Read the model definition and answer for the solid it produces. Units are mm, in the model's axes. Give positions to 0.01 mm unless a question says otherwise; leave off trailing zeros. Order: outer loops, then holes, each group sorted by start corner. A loop starts at its lowest first (then second) coordinate and runs counter-clockwise, first axis right, second up. Notation, with made-up numbers: (-30.5, 50.25) - (6.5, 50.25) arc R20 ccw to (6.5, 70.25) - close; hole circle Ø9 at (6.5, 1.5). An arc over 180 degrees is marked (long way). Use a Markdown table: item, result. Add a question column.
1. A cutting plane is placed at C-C on y = -22.5. Determine the outline of the cut face in (x, z).
2. A cutting plane is placed at B-B on y = -14. Determine the outline of the cut face in (x, z).
3. A cutting plane is placed at D-D on x = 8.5. Determine the outline of the cut face in (y, z).
4. A flat-ended cylindrical pin translates along its axis: P1, Ø0.6, axis at y = -22.5, z = 1.5, coming from the +X side. Find the tip coordinate at first contact, or state that the pin passes through.
5. A cutting plane is placed at A-A on z = 1.65. Determine the outline of the cut face in (x, y), and give its area (3 significant figures).
6. Consider L1, parallel to Y at x = 8.5, z = 1.55; L2, parallel to X at y = -17, z = 1.85; L3, parallel to Y at x = 6, z = 1.95. Determine where each line is inside the solid, lowest interval first.
```python
from build123d import *

# Parameters (mm, degrees)
SKETCH_1_R      = 2
EXTRUDE_1_DEPTH = 2


with BuildPart() as part:
    # 草图1 → 凸台-拉伸1 (new body)
    with BuildSketch(Plane.XY):
        with BuildLine():
            Line((-14.576201266, -23.207463353), (-15.742490369, -16.580463555))
            ThreePointArc((-15.742490369, -16.580463555), (-15.927700406, -16.024070615), (-16.26632367, -15.545311649))
            ThreePointArc((-16.26632367, -15.545311649), (0, 22.5), (16.26632367, -15.545311649))
            ThreePointArc((16.26632367, -15.545311649), (15.927700406, -16.024070615), (15.742490369, -16.580463555))
            Line((15.742490369, -16.580463555), (14.576201266, -23.207463353))
            ThreePointArc((14.576201266, -23.207463353), (14.420792767, -23.592708818), (14.122248494, -23.881563776))
            ThreePointArc((14.122248494, -23.881563776), (8.541490175, -26.531326793), (2.5, -27.822258212))
            Line((2.5, -27.822258212), (2.5, -19.67030278))
            ThreePointArc((2.5, -19.67030278), (0, 17.16), (-2.5, -19.67030278))
            Line((-2.5, -19.67030278), (-2.5, -27.822258212))
            ThreePointArc((-2.5, -27.822258212), (-8.541490175, -26.531326793), (-14.122248494, -23.881563776))
            ThreePointArc((-14.122248494, -23.881563776), (-14.420792767, -23.592708818), (-14.576201266, -23.207463353))
        make_face()
        with Locations((-8.5, -22.5)):
            Circle(SKETCH_1_R, mode=Mode.SUBTRACT)
        with Locations((8.5, -22.5)):
            Circle(SKETCH_1_R, mode=Mode.SUBTRACT)
    extrude(amount=EXTRUDE_1_DEPTH)


solid = part.part
```
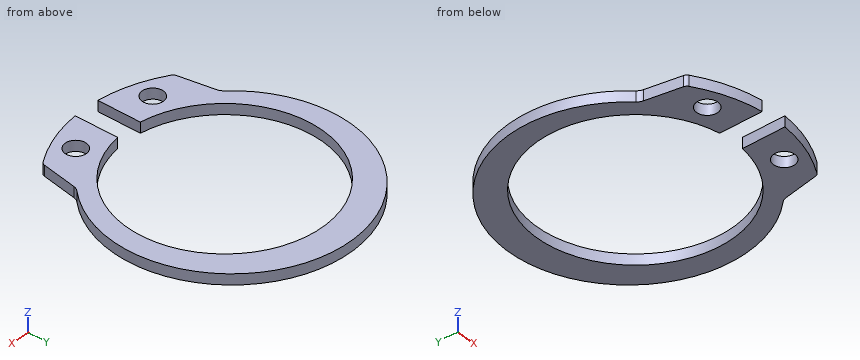
Output values:
| question | item | result |
|---|---|---|
| 1 | outline | (-14.7, 0) - (-10.5, 0) - (-10.5, 2) - (-14.7, 2) - close; (-6.5, 0) - (-2.5, 0) - (-2.5, 2) - (-6.5, 2) - close; (2.5, 0) - (6.5, 0) - (6.5, 2) - (2.5, 2) - close; (10.5, 0) - (14.7, 0) - (14.7, 2) - (10.5, 2) - close |
| 2 | outline | (-17.61, 0) - (-13.49, 0) - (-13.49, 2) - (-17.61, 2) - close; (13.49, 0) - (17.61, 0) - (17.61, 2) - (13.49, 2) - close |
| 3 | outline | (-26.55, 0) - (-24.5, 0) - (-24.5, 2) - (-26.55, 2) - close; (-20.5, 0) - (-17.77, 0) - (-17.77, 2) - (-20.5, 2) - close; (15.09, 0) - (20.83, 0) - (20.83, 2) - (15.09, 2) - close |
| 4 | P1 | x = 14.75 |
| 5 | outline | (-16.27, -15.55) arc R2 cw to (-15.74, -16.58) - (-14.58, -23.21) arc R1 ccw to (-14.12, -23.88) arc R26.6 ccw to (-2.5, -27.82) - (-2.5, -19.67) arc R18.5 cw (long way) to (2.5, -19.67) - (2.5, -27.82) arc R26.6 ccw to (14.12, -23.88) arc R1 ccw to (14.58, -23.21) - (15.74, -16.58) arc R2 cw to (16.27, -15.55) arc R22.5 ccw (long way) to start; hole circle Ø4 at (-8.5, -22.5); hole circle Ø4 at (8.5, -22.5) |
| 5 | area | 624 mm² |
| 6 | L1 | -26.55 to -24.5, -20.5 to -17.77, 15.09 to 20.83 |
| 6 | L2 | -15.67 to -9.85, 9.85 to 15.67 |
| 6 | L3 | -27.25 to -18.84, 16.16 to 21.69 |
